Geometry: final body of the model. Coordinates: model frame, mm. A direction names the side the tool comes from. Give positions to 0.01 mm unless a question says otherwise; leave off trailing zeros. Order: outer loops, then holes, each group sorted by start corner. A loop starts at its lowest first (then second) coordinate and runs counter-clockwise, first axis right, second up. Notation, with made-up numbers: (38, -11.5) -> (76, -11.5) arc R15 cw to (76, 5.5) -> close; hole circle Ø8 at (6, -9.5). An arc over 180 degrees is marked (long way). One line per question, with ' | ' between items.
from build123d import *

# Parameters (mm, degrees)
CUT_EXTRUDE_1_DEPTH = 4
CUT_EXTRUDE_START   = -1.3
SKETCH_3_R          = 15
SKETCH_3_R_2        = 14.3
CUT_EXTRUDE_2_DEPTH = 1.3
CUT_EXTRUDE_3_DEPTH = 4
SKETCH_5_R          = 15
SKETCH_5_R_2        = 14.3
CUT_EXTRUDE_4_DEPTH = 1.3


with BuildPart() as part:
    # 草图1 → 旋转1 (revolve)
    with BuildSketch(Plane.XY, mode=Mode.PRIVATE) as revolve_1_sk:
        Polygon((0, 0), (0, 15), (78, 15), (78, 17.5), (226, 17.5), (226, 25), (236, 25), (236, 60), (1086, 60), (1086, 25), (1096, 25), (1096, 17.5), (1229, 17.5), (1229, 15), (1261, 15), (1261, 0), align=None)
    revolve(revolve_1_sk.sketch.rotate(Axis((0, 0, 0), (1, 0, 0)), 90), axis=Axis((0, 0, 0), (1, 0, 0)))

    # 草图2 → 切除-拉伸1 (cut)
    with BuildSketch(Plane(origin=(0, 15, 0), x_dir=(1, 0, 0), z_dir=(0, 1, 0))):
        with BuildLine():
            Line((68, 4), (-10, 4))
            Line((-10, 4), (-10, -4))
            Line((-10, -4), (68, -4))
            ThreePointArc((68, -4), (72, 0), (68, 4))
        make_face()
    extrude(amount=-CUT_EXTRUDE_1_DEPTH, mode=Mode.SUBTRACT)

    # 草图3 → 切除-拉伸2 (cut)
    with BuildSketch(Plane.ZY.offset(-12.8).offset(CUT_EXTRUDE_START)):
        Circle(SKETCH_3_R)
        Circle(SKETCH_3_R_2, mode=Mode.SUBTRACT)
    extrude(amount=CUT_EXTRUDE_2_DEPTH, mode=Mode.SUBTRACT)

    # 草图4 → 切除-拉伸3 (cut)
    with BuildSketch(Plane(origin=(0, 15, 0), x_dir=(1, 0, 0), z_dir=(0, 1, 0))):
        with BuildLine():
            Line((1239, 4), (1271, 4))
            Line((1271, 4), (1271, -4))
            Line((1271, -4), (1239, -4))
            ThreePointArc((1239, -4), (1235, 0), (1239, 4))
        make_face()
    extrude(amount=-CUT_EXTRUDE_3_DEPTH, mode=Mode.SUBTRACT)

    # 草图5 → 切除-拉伸4 (cut)
    with BuildSketch(Plane(origin=(1248.2, 0, 0), x_dir=(0, 0, -1), z_dir=(1, 0, 0))):
        with Locations(Location((0, 0, 0), (0, 0, 180))):
            Circle(SKETCH_5_R)
        Circle(SKETCH_5_R_2, mode=Mode.SUBTRACT)
    extrude(amount=-CUT_EXTRUDE_4_DEPTH, mode=Mode.SUBTRACT)


solid = part.part
1) Set-up query: faces 4 (the cylindrical face through (1238.08, -12.65, 8.06)), 5 (the flat face through (1246.9, -13.4, -5.6)), 6 (the flat face through (226, 5, 17)). Return all of +Z, -Z, +X, -X, +Y, -Y with unobstructed straight access to the full face (end or side cutting, diameter ignored); none if empty.
Check result:
face 4: +X | face 5: none | face 6: -X
2) Section B-B on y = 42. Return loops of the section in (x, z), plus the area to 3 significant figures.
Check result:
outline: (236, -42.85) -> (1086, -42.85) -> (1086, 42.85) -> (236, 42.85) -> close | area: 72,800 mm^2
3) Section A-A on x = 308. Return loops of the section in (y, z), plus the area to 3 significant figures.
Check result:
outline: circle Ø120 at (0, 0) | area: 11,300 mm^2
4) Contact query for flat-ended pins moving along their axis: pin 1 Ø3 at (x, y) = (1250.5, 12.5) entering from -Z; pin 2 Ø25 at (y, z) = (-3, -12.5) entering from -X; pin 3 Ø4 at (x, y) = (1246, 12.5) entering from +Z; pin 4 Ø1 at (x, y) = (236.5, 9.5) entering from -Z. Output: stop coordinate, or through.
Check result:
pin 1: stops at z = -10.2 | pin 2: stops at x = 0 | pin 3: stops at z = 10.71 | pin 4: stops at z = -59.32
5) Pull-direction query (X, two-part tool) for faces 1 (the flat face through (12.8, -14.4, 2.2)), 2 (the cylindrical face through (153.036, 17.084, -3.794)), 3 (the flat face through (78, -8, -13)); classes: +X half, -X half, draft (parallel to the pull), parting line (faces both ways), or undercut.
Check result:
face 1: undercut | face 2: draft | face 3: -X half
6) Material intervals for probe 1 along X at (y, z) = (-31.5, -24.5); probe 2 along Y at (x, z) = (313.5, 5); probe 3 along Y at (x, z) = (1138, -10), sorted ascending. Write a range as from..to.
Check result:
probe 1: x = 236..1086 | probe 2: y = -59.79..59.79 | probe 3: y = -14.36..14.36
7) Section C-C on z = -36.5. Return loops of the section in (x, y).
Check result:
outline: (236, -47.62) -> (1086, -47.62) -> (1086, 47.62) -> (236, 47.62) -> close
